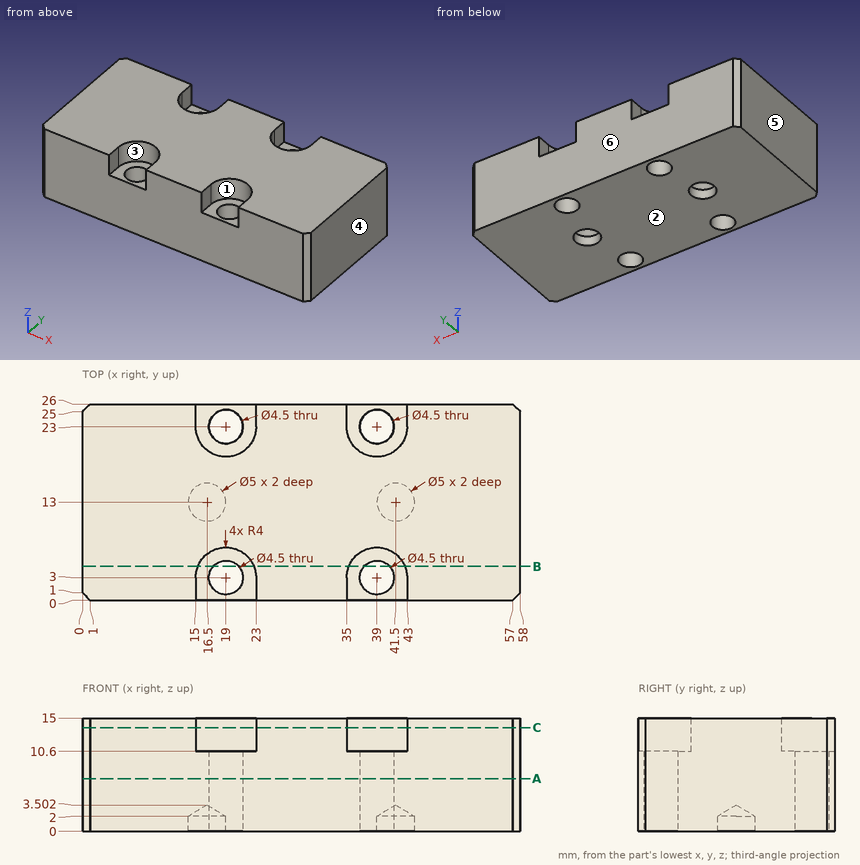
Design review of the part shown in the three views and the two pictorial views. Dimensions are in mm from the part's minimum x, y and z. A direction names the side the tool comes from. Give positions to 0.01 mm unless a question says otherwise; leave off trailing zeros. Write each loop counter-clockwise with the first axis right and the second up, starting at its lowest first coordinate (ties: lowest second). Pieces come first, ordered by that corner, then holes. Notation, with made-up numbers: M 66,50 L 107,50 A32 ccw 107,83 Z; hole C 80.25,26 d6. An arc over 180 degrees is marked long. Return JSON: item names as keys, results as strings. Group by question number.
Item 1: Tool access review of the marked faces 1 and 2: name each direction out of +Z, -Z, +X, -X, +Y, -Y from which nothing blocks a thin tool from reaching the whole face with its end or side.
Item 2: Wall thickness on line 1 along Y through (x, z) = (39, 7); line 2 along Y through (x, z) = (41.5, 0.6); line 3 along X through (y, z) = (24, 3.75) (1 decimal): over which ranges is each line inside the solid? List them lowest first.
Item 3: The part is to be moulded in two halves that separate along X. For the marked faces 3, 4, 5 and 6, say which applies: pulls with the +X half, pulls with the -X half, needs draft (parallel to the pull), parting line crosses it, or undercut.
Item 4: Take a section at A-A (z = 7). Give the boundary of the cut face in (x, y).
Item 5: Take a section at C-C (z = 13.75). Give the boundary of the cut face in (x, y), plus the area to 3 significant figures.
Item 6: Take a section at B-B (y = 4.5). Give the boundary of the cut face in (x, z), plus the area to 3 significant figures.
Item 7: Clearance check with flat-ended pins moving along their axes: pin 1 Ø8 at (x, y) = (41.5, 13) entering from -Z; pin 2 Ø3.5 at (x, y) = (17, 3.5) entering from +Z; pin 3 Ø3 at (x, y) = (16.5, 13) entering from -Z. State where each tip first meets the part, or that it passes through.
Return value:
{
 "1": {"face 1": "+Z, -Y", "face 2": "-Z, +X, -X, +Y, -Y"},
 "2": {"line 1": "y = 0 to 0.75, 5.25 to 20.75, 25.25 to 26", "line 2": "y = 0 to 10.5, 15.5 to 26", "line 3": "x = 0 to 17, 21 to 37, 41 to 58"},
 "3": {"face 3": "undercut", "face 4": "pulls with the +X half", "face 5": "pulls with the -X half", "face 6": "needs draft"},
 "4": {"outline": "M 0,1 L 1,0 L 57,0 L 58,1 L 58,25 L 57,26 L 1,26 L 0,25 Z; hole C 19,3 d4.5; hole C 19,23 d4.5; hole C 39,3 d4.5; hole C 39,23 d4.5"},
 "5": {"outline": "M 0,1 L 1,0 L 15,0 L 15,3 A4 cw 23,3 L 23,0 L 35,0 L 35,3 A4 cw 43,3 L 43,0 L 57,0 L 58,1 L 58,25 L 57,26 L 43,26 L 43,23 A4 cw 35,23 L 35,26 L 23,26 L 23,23 A4 cw 15,23 L 15,26 L 1,26 L 0,25 Z", "area": "1,310 mm2"},
 "6": {"outline": "M 0,0 L 17.32,0 L 17.32,10.6 L 15.29,10.6 L 15.29,15 L 0,15 Z; M 20.68,0 L 37.32,0 L 37.32,10.6 L 35.29,10.6 L 35.29,15 L 22.71,15 L 22.71,10.6 L 20.68,10.6 Z; M 40.68,0 L 58,0 L 58,15 L 42.71,15 L 42.71,10.6 L 40.68,10.6 Z", "area": "734 mm2"},
 "7": {"pin 1": "stops at z = 0", "pin 2": "stops at z = 10.6", "pin 3": "stops at z = 2.6"}
}
